from build123d import *

# Parameters (mm, degrees)
BASE_BLOCK_DEPTH    = 50
ROUND_BOSS_SKETCH_R = 20
ROUND_BOSS_DEPTH    = 15
TOP_KEY_SKETCH_W    = 40
TOP_KEY_SKETCH_H    = 16
TOP_KEY_DEPTH       = 15
SLOT_SKETCH_W       = 30
SLOT_SKETCH_H       = 29
SLOT_CUT_DEPTH      = 15


with BuildPart() as part:
    # Base Profile Sketch → Base Block (new body)
    with BuildSketch(Plane.XY):
        Polygon((15, -5), (45, -5), (45, 5), (-45, 5), (-45, -5), (-15, -5), (-15, -15), (15, -15), align=None)
    extrude(amount=BASE_BLOCK_DEPTH)

    # Loft Top Profile Sketch → section 0 of tapered_body_loft
    with BuildSketch(Plane(origin=(0, 55, 0), x_dir=(1, 0, 0), z_dir=(0, 1, 0)), mode=Mode.PRIVATE) as tapered_body_loft_s0:
        with BuildLine():
            Line((-25, 0), (25, 0))
            Line((25, 0), (25, -50))
            Line((25, -50), (-25, -50))
            Line((-25, -50), (-25, 0))
        make_face()
    # loft up to a face of the part (tapered_body_loft)
    loft([tapered_body_loft_s0.sketch, part.faces().sort_by_distance((0, 5, 25))[0]])

    # Round Boss Sketch → Round Boss (add)
    with BuildSketch(Plane(origin=(0, 55, 0), x_dir=(1, 0, 0), z_dir=(0, 1, 0))):
        with Locations(Location((0, -25, 0), (0, 0, 270))):
            Circle(ROUND_BOSS_SKETCH_R)
    extrude(amount=ROUND_BOSS_DEPTH)

    # Top Key Sketch → Top Key (add)
    with BuildSketch(Plane(origin=(0, 70, 0), x_dir=(1, 0, 0), z_dir=(0, 1, 0))):
        with Locations((0, -25)):
            Rectangle(TOP_KEY_SKETCH_W, TOP_KEY_SKETCH_H)
    extrude(amount=TOP_KEY_DEPTH)

    # Slot Sketch → Slot Cut (cut)
    with BuildSketch(Plane(origin=(-40.517241379, 16.206896552, 0), x_dir=(0, 0, 1), z_dir=(-0.9284766908852594, 0.37139067635410355, 0))):
        with Locations((25, 16.28145109)):
            Rectangle(SLOT_SKETCH_W, SLOT_SKETCH_H)
    extrude(amount=-SLOT_CUT_DEPTH, mode=Mode.SUBTRACT)


solid = part.part
Build history of the part. All positions in model axes, mm. A direction names the side the tool comes from. Coordinates: 2 decimals unless noted, no trailing zeros. Order: outer loops, then holes, each group sorted by start corner. A loop starts at its lowest first (then second) coordinate and runs counter-clockwise, first axis right, second up. Notation, with made-up numbers: (-2, 68) - (47, 68) arc R13 ccw to (47, 74) - close; hole circle Ø10 at (40.25, 52.25). An arc over 180 degrees is marked (long way). Write item = value, one per line. Start each with the question number.
1) 3-axis set-ups, long thin cutter, end or side, ignore diameter. For faces 4 (the face through (-15, -10, 25)), 5 (the face through (6.007, 62.395, 44.076)), 6 (the face through (0, 77, 17)), 7 (the face through (0, 70, 38)): which of +Z, -Z, +X, -X, +Y, -Y reach the whole face in a straight line?
2) Saw through at D-D on y = 37.5. Write the cut outline in (x, z), then the cut area to 3 significant figures.
3) Wall check: line 1 along X through (y, z) = (-9.5, 3); line 2 along Y through (x, z) = (14.5, 10.5); line 3 along Z through (x, y) = (9, 72). Give the ranges that are in metal, low to high. Write a range as from..to.
4) Flat gauge pins, fed straight in: pin 1 Ø5 at (x, z) = (-35, 14.5) entering from +Y; pin 2 Ø0.5 at (x, z) = (-19.5, 29) entering from -Y; pin 3 Ø20 at (x, y) = (-27, 23) entering from -Z; pin 4 Ø1 at (x, y) = (-13.5, 57.5) entering from -Z. Where does each tip first touch, or does it go through?
5) Saw through at B-B on z = 22. Write the cut outline in (x, y).
6) Two-plate mould, pull along X, no slides. Class faces 1 (the face through (0, 70, 12)), 2 (the face through (20, 77, 25)), 3 (the face through (-20.47, 25.94, 24.79)): pulls with the +X half, pulls with the -X half, needs draft (parallel to the pull), parting line crosses it, or undercut.
7) Saw through at A-A on x = -23. Write the cut outline in (y, z), then the cut area to 3 significant figures.
8) Saw through at C-C on x = 0. Write the cut outline in (y, z), then the cut area to 3 significant figures.
From the geometry:
q1.face_4 = +Z, -Z, -X, -Y
q1.face_5 = none
q1.face_6 = -Z, +X, -X, +Y
q1.face_7 = +Z, +X, -X, +Y
q2.outline = (-32, 0) - (32, 0) - (32, 50) - (-32, 50) - (-32, 40) - (-15.84, 40) - (-15.84, 10) - (-32, 10) - close
q2.area = 2,720 mm^2
q3.line_1 = -15..15
q3.line_2 = -15..55
q3.line_3 = 17..33
q4.pin_1 = 16.92
q4.pin_2 = -5
q4.pin_3 = 0
q4.pin_4 = 9.8
q5.outline = (-45, -5) - (-15, -5) - (-15, -15) - (15, -15) - (15, -5) - (45, -5) - (45, 5) - (25, 55) - (19.77, 55) - (19.77, 70) - (20, 70) - (20, 85) - (-20, 85) - (-20, 70) - (-19.77, 70) - (-19.77, 55) - (-25, 55) - (-29.09, 44.79) - (-15.16, 39.22) - (-25.93, 12.29) - (-39.86, 17.86) - (-45, 5) - close
q6.face_1 = needs draft
q6.face_2 = pulls with the +X half
q6.face_3 = undercut
q7.outline = (-5, 0) - (55, 0) - (55, 50) - (-5, 50) - close; hole (19.61, 10) - (42.35, 10) - (42.35, 40) - (19.61, 40) - close
q7.area = 2,320 mm^2
q8.outline = (-15, 0) - (55, 0) - (55, 5) - (70, 5) - (70, 17) - (85, 17) - (85, 33) - (70, 33) - (70, 45) - (55, 45) - (55, 50) - (-15, 50) - close
q8.area = 4,340 mm^2
